Check sheet for the modelled part. Datum: model origin and axes. Units: mm. Give positions to 0.01 mm unless a question says otherwise; leave off trailing zeros. Order: outer loops, then holes, each group sorted by start corner. A loop starts at its lowest first (then second) coordinate and runs counter-clockwise, first axis right, second up.
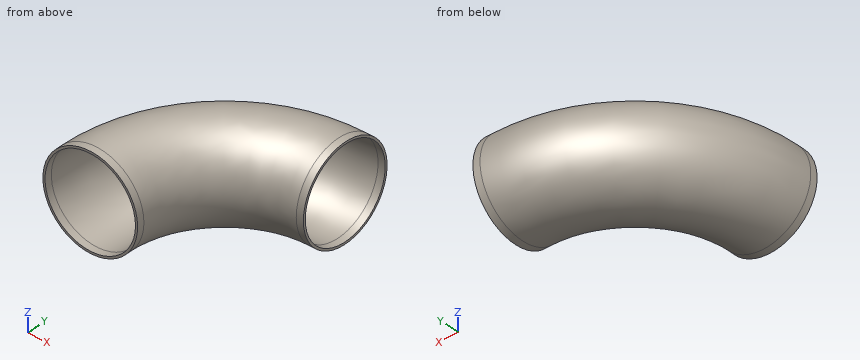
```python
from build123d import *

# Parameters (mm, degrees)
SKETCH1_R = 66.5
SHELL1_T  = -3


with BuildPart() as part:
    # Sweep1: sweep along a path in Sketch2
    with BuildLine(Plane.XY) as sweep1_path:
        Line((0, 0), (0, 10))
        ThreePointArc((0, 10), (52.720779386, 137.279220614), (180, 190))
        Line((180, 190), (190, 190))
    # Sketch1 → Sweep1 (sweep)
    with BuildSketch(Plane(origin=(0, 0, 0), x_dir=(1, 0, 0), z_dir=(0, 1, 0))):
        Circle(SKETCH1_R)
    sweep(path=sweep1_path.line)

    # Shell1
    shell1_openings = [part.faces().sort_by_distance(p)[0] for p in [
        (190, 190, 0),
        (0, 0, 0),
    ]]
    offset(amount=SHELL1_T, openings=shell1_openings, kind=Kind.INTERSECTION)


solid = part.part
```
(1) Go/stop test with flat-tipped pins: P1, Ø5, axis at x = 46.5, z = 50, coming from the +Y side; P2, Ø2, axis at y = 221, z = 19, coming from the -X side; P3, Ø6, axis at y = 34.5, z = -47, coming from the +X side. Record where each tip stops, or that it passes through.
(2) Thickness scan on L1, parallel to X at y = 4.5, z = 0; L2, parallel to X at y = 48.5, z = 52. Record the ranges inside material, lowest first.
(3) Sectioned sample at A-A (z = 0). Enter the section's corners in (x, y).
(4) Sectioned sample at B-B (z = -15.5). Enter the section's corners in (x, y), plus the area to 3 significant figures.
Values follow:
1. P1: stops at y = 193.51
1. P2: stops at x = 56.2
1. P3: stops at x = 52.25
2. L1: x = -66.5 to -63.5, 63.5 to 66.5
2. L2: x = -38.08 to -32.99, 41.7 to 46.91
3. outline: (-66.5, 0) - (-63.5, 0) - (-63.5, 10) arc R243.5 cw to (180, 253.5) - (190, 253.5) - (190, 256.5) - (180, 256.5) arc R246.5 ccw to (-66.5, 10) - close; (63.5, 0) - (66.5, 0) - (66.5, 10) arc R113.5 cw to (180, 123.5) - (190, 123.5) - (190, 126.5) - (180, 126.5) arc R116.5 ccw to (63.5, 10) - close
4. outline: (-64.67, 0) - (-61.58, 0) - (-61.58, 10) arc R241.58 cw to (180, 251.58) - (190, 251.58) - (190, 254.67) - (180, 254.67) arc R244.67 ccw to (-64.67, 10) - close; (61.58, 0) - (64.67, 0) - (64.67, 10) arc R115.33 cw to (180, 125.33) - (190, 125.33) - (190, 128.42) - (180, 128.42) arc R118.42 ccw to (61.58, 10) - close
4. area: 1,870 mm2
